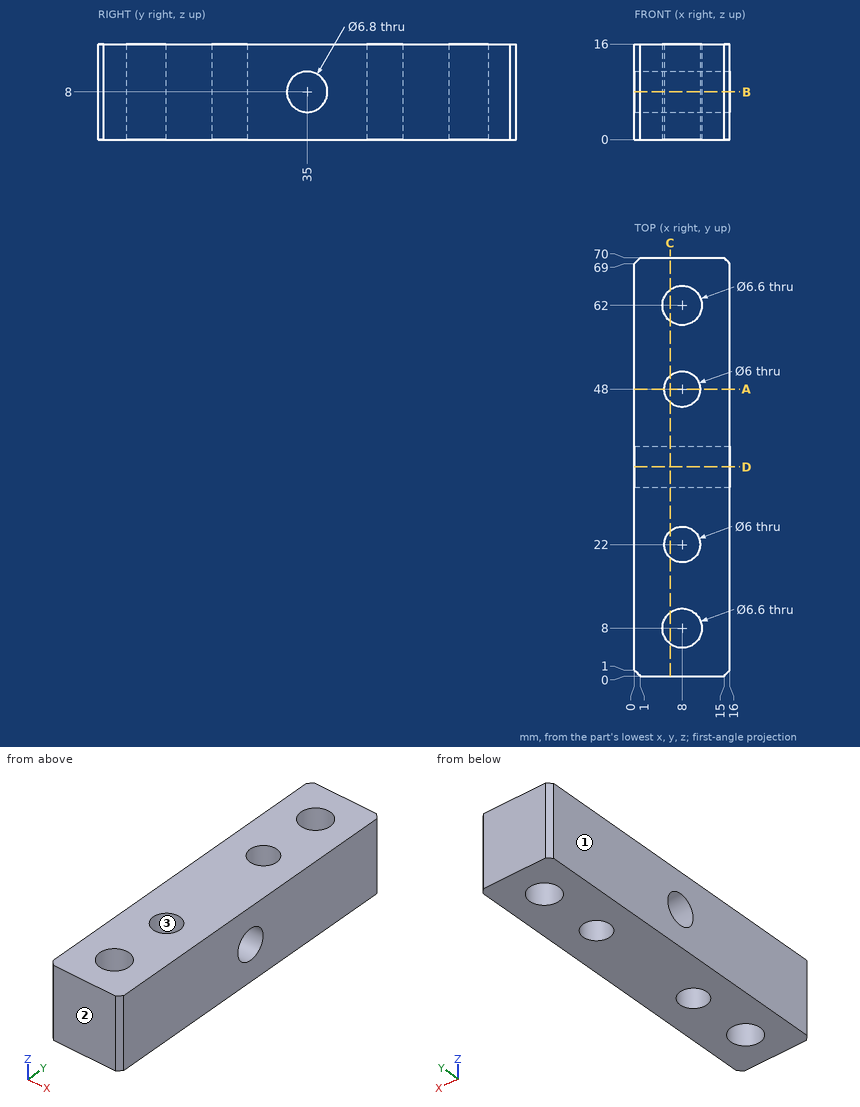
Part print with two shaded views. Sizes in mm from the minimum x, y, z corner. Coordinates: 2 decimals unless noted, no trailing zeros. Write each loop counter-clockwise with the first axis right and the second up, starting at its lowest first coordinate (ties: lowest second). Pieces come first, ordered by that corner, then holes.
1. Drill centre lines: probe 1 along Y at (x, z) = (8, 3.5); probe 2 along Y at (x, z) = (8, 5); probe 3 along Y at (x, z) = (5.5, 7). Where is each one in solid material? Low to high.
Answer block:
probe 1: y = 0 to 4.7, 11.3 to 19, 25 to 45, 51 to 58.7, 65.3 to 70
probe 2: y = 0 to 4.7, 11.3 to 19, 25 to 33.4, 36.6 to 45, 51 to 58.7, 65.3 to 70
probe 3: y = 0 to 5.85, 10.15 to 20.34, 23.66 to 31.75, 38.25 to 46.34, 49.66 to 59.85, 64.15 to 70
2. Band-saw the part on D-D, the plane y = 35. Give the cut face in (x, z), and give its area (3 significant figures).
Answer block:
outline: (0, 0) - (16, 0) - (16, 4.6) - (0, 4.6) - close; (0, 11.4) - (16, 11.4) - (16, 16) - (0, 16) - close
area: 147 mm2
3. Pull direction Y, two halves, no side cores. Call the marked faces 1, 2 and 3: released by +Y, released by -Y, zero draft, split by the parting line, or undercut.
Answer block:
face 1: zero draft
face 2: released by -Y
face 3: undercut
4. Band-saw the part on B-B, the plane z = 8. Give the cut face in (x, y).
Answer block:
outline: (0, 1) - (1, 0) - (15, 0) - (16, 1) - (16, 31.6) - (0, 31.6) - close; (0, 38.4) - (16, 38.4) - (16, 69) - (15, 70) - (1, 70) - (0, 69) - close; hole circle Ø6.6 at (8, 8); hole circle Ø6.6 at (8, 62); hole circle Ø6 at (8, 22); hole circle Ø6 at (8, 48)
5. Band-saw the part on C-C, the plane x = 6. Give the cut face in (y, z), and give its area (3 significant figures).
Answer block:
outline: (0, 0) - (5.38, 0) - (5.38, 16) - (0, 16) - close; (10.62, 0) - (19.76, 0) - (19.76, 16) - (10.62, 16) - close; (24.24, 0) - (45.76, 0) - (45.76, 16) - (24.24, 16) - close; (50.24, 0) - (59.38, 0) - (59.38, 16) - (50.24, 16) - close; (64.62, 0) - (70, 0) - (70, 16) - (64.62, 16) - close; hole circle Ø6.8 at (35, 8)
area: 773 mm2
6. Band-saw the part on A-A, the plane y = 48. Give the cut face in (x, z), and give its area (3 significant figures).
Answer block:
outline: (0, 0) - (5, 0) - (5, 16) - (0, 16) - close; (11, 0) - (16, 0) - (16, 16) - (11, 16) - close
area: 160 mm2
7. Drop a flat-ended pin along its axis: pin 1 (8 mm diameter, centred on x = 8.5, y = 8, fed in from +Z). Give the stop position or say it passes through.
Answer block:
pin 1: stops at z = 16
